Here's how the part is built. I have some questions about the finished solid (model axes, mm). Face numbers are marked on the shaded views. A direction names the side the tool comes from. Give positions to 0.01 mm unless a question says otherwise; leave off trailing zeros. Write each loop counter-clockwise with the first axis right and the second up, starting at its lowest first coordinate (ties: lowest second). Pieces come first, ordered by that corner, then holes. Notation, with made-up numbers: (62, 18) - (97, 18) arc R12 cw to (97, 34) - close; hole circle Ø9 at (-9.75, 48). An arc over 180 degrees is marked (long way). One line per item, written item: value. Start each with the question number.
1) Imagine slicing it at B-B on x = 0.5. Write out the boundary of the cut face in (y, z).
2) I'm going to push a flat-ended pin straight in: P1, Ø1.5, axis at y = 183, z = -18.5, coming from the -X side. Where does the tip first touch, or does it pass through?
3) On a 3-axis mill with a long thin cutter (end or side, diameter ignored), from which of +Z, -Z, +X, -X, +Y, -Y can I reach the whole of each face in a straight line? I mean the marked faces 1 and 2. Say none if no direction works.
4) We'd pull the mould along X, two halves only. Please class the marked faces 3, 4 and 5: +X half, -X half, draft (parallel to the pull), parting line (faces both ways), or undercut.
5) Imagine slicing it at A-A on y = 117.5. Write out the boundary of the cut face in (x, z).
6) Imagine slicing it at C-C on z = -10. Write out the boundary of the cut face in (x, y), plus the area to 3 significant figures.
7) Please list where these lines run through material, in increasing order: L1, parallel to X at y = 86.5, z = 4; L2, parallel to X at y = 180.5, z = 16. Write a range as [from, to].
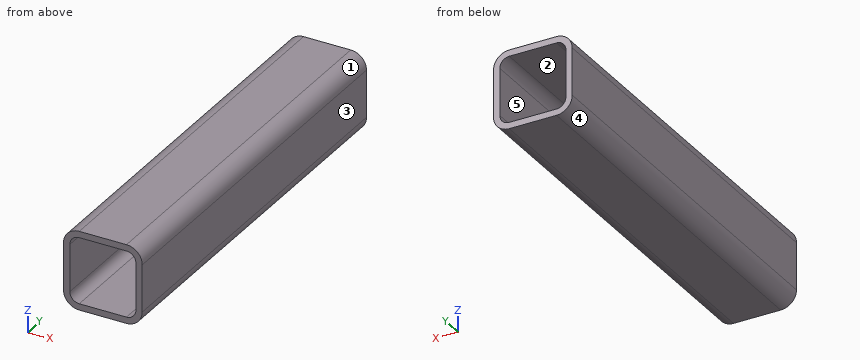
from build123d import *

# Parameters (mm, degrees)
BOSS_EXTRUDE1_DEPTH = 250


with BuildPart() as part:
    # Sketch1 → Boss-Extrude1 (new body)
    with BuildSketch(Plane(origin=(0, 0, 0), x_dir=(1, 0, 0), z_dir=(0, 1, 0))):
        with BuildLine():
            Line((-15, -25), (15, -25))
            ThreePointArc((15, -25), (22.071067812, -22.071067812), (25, -15))
            Line((25, -15), (25, 15))
            ThreePointArc((25, 15), (22.071067812, 22.071067812), (15, 25))
            Line((15, 25), (-15, 25))
            ThreePointArc((-15, 25), (-22.071067812, 22.071067812), (-25, 15))
            Line((-25, 15), (-25, -15))
            ThreePointArc((-25, -15), (-22.071067812, -22.071067812), (-15, -25))
        make_face()
        with BuildLine():
            Line((-15, 21), (15, 21))
            ThreePointArc((15, 21), (19.242640687, 19.242640687), (21, 15))
            Line((21, 15), (21, -15))
            ThreePointArc((21, -15), (19.242640687, -19.242640687), (15, -21))
            Line((15, -21), (-15, -21))
            ThreePointArc((-15, -21), (-19.242640687, -19.242640687), (-21, -15))
            Line((-21, -15), (-21, 15))
            ThreePointArc((-21, 15), (-19.242640687, 19.242640687), (-15, 21))
        make_face(mode=Mode.SUBTRACT)
    extrude(amount=BOSS_EXTRUDE1_DEPTH)


solid = part.part
Numbers:
1. outline: (0, -25) - (250, -25) - (250, -21) - (0, -21) - close; (0, 21) - (250, 21) - (250, 25) - (0, 25) - close
2. P1: x = -24.61
3. face 1: +Z, +X, +Y, -Y
3. face 2: +Y, -Y
4. face 3: +X half
4. face 4: -X half
4. face 5: undercut
5. outline: (-25, -15) arc R10 ccw to (-15, -25) - (15, -25) arc R10 ccw to (25, -15) - (25, 15) arc R10 ccw to (15, 25) - (-15, 25) arc R10 ccw to (-25, 15) - close; hole (-21, -15) arc R6 ccw to (-15, -21) - (15, -21) arc R6 ccw to (21, -15) - (21, 15) arc R6 ccw to (15, 21) - (-15, 21) arc R6 ccw to (-21, 15) - close
6. outline: (-25, 0) - (-21, 0) - (-21, 250) - (-25, 250) - close; (21, 0) - (25, 0) - (25, 250) - (21, 250) - close
6. area: 2,000 mm^2
7. L1: [-25, -21], [21, 25]
7. L2: [-24.95, -20.92], [20.92, 24.95]
